```python
from build123d import *

# Parameters (mm, degrees)
EXTRUDE_1_DEPTH = 3


with BuildPart() as part:
    # 草图1 → 凸台-拉伸1 (new body)
    with BuildSketch(Plane.XY):
        Polygon((-25.609151467, -21.768855911), (-20.609151467, -21.768855911), (-20.609151467, -24.768855911), (-10.609151467, -24.768855911), (-10.609151467, -21.768855911), (9.390848533, -21.768855911), (9.390848533, -24.768855911), (19.390848533, -24.768855911), (19.390848533, -21.768855911), (24.390848533, -21.768855911), (24.390848533, -12.618855911), (11.890848533, -7.618855911), (11.890848533, 7.381144089), (24.390848533, 12.381144089), (24.390848533, 21.531144089), (19.390848533, 21.531144089), (19.390848533, 24.531144089), (9.390848533, 24.531144089), (9.390848533, 21.531144089), (-10.609151467, 21.531144089), (-10.609151467, 24.531144089), (-20.609151467, 24.531144089), (-20.609151467, 21.531144089), (-25.609151467, 21.531144089), (-25.609151467, 12.381144089), (-13.109151467, 7.381144089), (-13.109151467, -7.618855911), (-25.609151467, -12.618855911), align=None)
        with BuildLine():
            Line((1.890848533, 8.631144089), (1.890848533, -8.868855911))
            ThreePointArc((1.890848533, -8.868855911), (-0.609151467, -11.368855911), (-3.109151467, -8.868855911))
            Line((-3.109151467, -8.868855911), (-3.109151467, 8.631144089))
            ThreePointArc((-3.109151467, 8.631144089), (-0.609151467, 11.131144089), (1.890848533, 8.631144089))
        make_face(mode=Mode.SUBTRACT)
    extrude(amount=EXTRUDE_1_DEPTH)


solid = part.part
```
Verification items for the finished model (mm, model axes). A direction names the side the tool comes from. Coordinates: 2 decimals unless noted, no trailing zeros. Loops run counter-clockwise (first coordinate to the right, second up) from the corner with the lowest first, then second, coordinate; pieces in that order, holes last. Notation, with made-up numbers: (68, 6) - (75, 6) arc R34 ccw to (75, 41) - close; hole circle Ø6 at (17, 32.25). An arc over 180 degrees is marked (long way). Answer as a JSON object with one key per item and string values.
(1) Mould release check, pull along X, two halves, no side actions. Record for faces 1 (the flat face through (-19.447, 9.916, 1.479)), 2 (the flat face through (0, 21.531, 1)), 3 (the flat face through (18.053, 9.846, 1.479)): pulls with the +X half, pulls with the -X half, needs draft (parallel to the pull), parting line crosses it, or undercut.
Response:
{"face 1": "pulls with the -X half", "face 2": "undercut", "face 3": "pulls with the +X half"}
(2) Access from +Z, -Z, +X, -X, +Y, -Y to the whole of each face (thin tool, end or side, straight path). Record for faces 4 (the cylindrical face through (-0.66, 11.13, 1.48)), 5 (the flat face through (22, -21.769, 1)), 6 (the flat face through (19.391, 23, 1)).
Response:
{"face 4": "+Z, -Z", "face 5": "+Z, -Z, +X, -Y", "face 6": "+Z, -Z, +X, +Y"}
(3) Scan lines: line 1 along X through (y, z) = (22.5, 1.7); line 2 along X through (y, z) = (6.5, 1.3); line 3 along Y through (x, z) = (16, 2.6). Record each from-to range of solid material in increasing order.
Response:
{"line 1": "x = -20.61 to -10.61, 9.39 to 19.39", "line 2": "x = -13.11 to -3.11, 1.89 to 11.89", "line 3": "y = -24.77 to -9.26, 9.02 to 24.53"}
(4) Cross-section at C-C, the plane x = 20.5. Record the boundary of the cut face in (y, z), then the cut area to 3 significant figures.
Response:
{"outline": "(-21.77, 0) - (-11.06, 0) - (-11.06, 3) - (-21.77, 3) - close; (10.82, 0) - (21.53, 0) - (21.53, 3) - (10.82, 3) - close", "area": "64.2 mm²"}
(5) Cross-section at D-D, the plane x = -8. Record the boundary of the cut face in (y, z).
Response:
{"outline": "(-21.77, 0) - (21.53, 0) - (21.53, 3) - (-21.77, 3) - close"}
(6) Cross-section at A-A, the plane y = -3. Record the boundary of the cut face in (x, z), then the cut area to 3 significant figures.
Response:
{"outline": "(-13.11, 0) - (-3.11, 0) - (-3.11, 3) - (-13.11, 3) - close; (1.89, 0) - (11.89, 0) - (11.89, 3) - (1.89, 3) - close", "area": "60.0 mm²"}
(7) Go/stop test with flat-tipped pins: pin 1 Ø0.9 at (y, z) = (23, 1) entering from -X; pin 2 Ø0.9 at (x, z) = (22, 1) entering from -Y; pin 3 Ø0.9 at (y, z) = (23, 1) entering from +X. Record where each tip stops, or that it passes through.
Response:
{"pin 1": "stops at x = -20.61", "pin 2": "stops at y = -21.77", "pin 3": "stops at x = 19.39"}
